Geometry: see drawing. Coordinates: mm, zero at the bounding-box minimum. A direction names the side the tool comes from. Coordinates: 2 decimals unless noted, no trailing zeros. Loops run counter-clockwise (first coordinate to the right, second up) from the corner with the lowest first, then second, coordinate; pieces in that order, holes last. Notation, with made-up numbers: (67.5, 78.5) - (98.5, 78.5) arc R20 cw to (98.5, 100.5) - close; hole circle Ø9 at (-20.75, -32). An arc over 180 degrees is marked (long way). Write item = value, one per line. Start each with the question number.
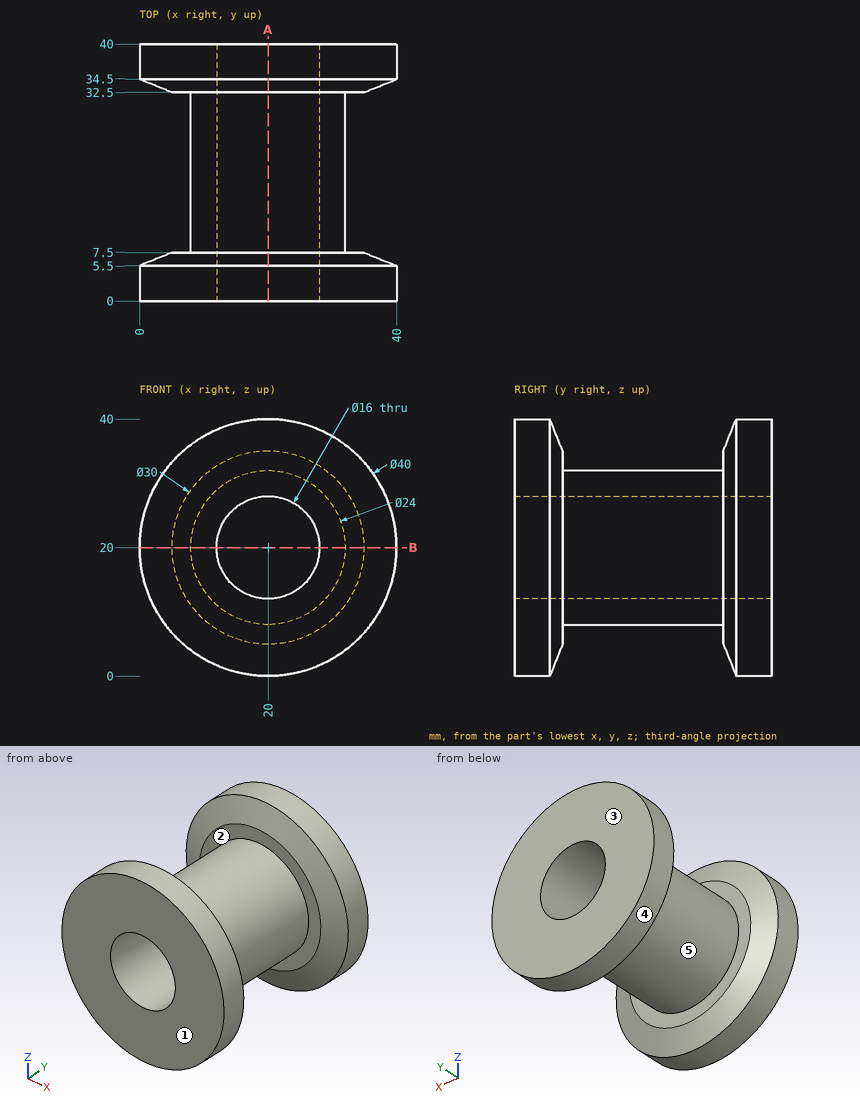
Item 1: Reachability of the marked faces 1 and 2 from +Z, -Z, +X, -X, +Y, -Y: full face, straight path, thin tool, end or side. Return the list, or none.
Item 2: Material intervals for L1, parallel to Y at x = 31, z = 25.5; L2, parallel to X at y = 15.5, z = 20; L3, parallel to Y at x = 38.5, z = 25, sorted ascending. Write a range as [from, to].
Item 3: Cut plane B-B (z = 20). Return the cut outline in (x, y), then the cut area to 3 significant figures.
Item 4: First-contact query: pin 1 (5 mm diameter, centred on y = 15, z = 7, fed in from +X); pin 2 (3 mm diameter, centred on y = 17.5, z = 23, fed in from +X); pin 3 (6 mm diameter, centred on x = 16, y = 16.5, fed in from +Z). Flat tips, straight axial feed; report the tip coordinate or a pass-through.
Item 5: Draft query along Y for the marked faces 3, 4 and 5. Return one class per face: released by +Y, released by -Y, zero draft, split by the parting line, or undercut.
Item 6: Cut plane A-A (x = 20). Return the cut outline in (y, z), then the cut area to 3 significant figures.
Responses:
q1.face_1 = +Z, -Z, +X, -X, -Y
q1.face_2 = none
q2.L1 = [0, 7.5], [32.5, 40]
q2.L2 = [8, 12], [28, 32]
q2.L3 = [0, 5.83], [34.17, 40]
q3.outline = (0, 0) - (12, 0) - (12, 40) - (0, 40) - (0, 34.5) - (5, 32.5) - (8, 32.5) - (8, 7.5) - (5, 7.5) - (0, 5.5) - close; (28, 0) - (40, 0) - (40, 5.5) - (35, 7.5) - (32, 7.5) - (32, 32.5) - (35, 32.5) - (40, 34.5) - (40, 40) - (28, 40) - close
q3.area = 540 mm2
q4.pin_1 = 25.81
q4.pin_2 = 31.91
q4.pin_3 = 31.96
q5.face_3 = released by +Y
q5.face_4 = zero draft
q5.face_5 = undercut
q6.outline = (0, 0) - (5.5, 0) - (7.5, 5) - (7.5, 8) - (32.5, 8) - (32.5, 5) - (34.5, 0) - (40, 0) - (40, 12) - (0, 12) - close; (0, 28) - (40, 28) - (40, 40) - (34.5, 40) - (32.5, 35) - (32.5, 32) - (7.5, 32) - (7.5, 35) - (5.5, 40) - (0, 40) - close
q6.area = 540 mm2
